Verification items for the finished model (mm, model axes). A direction names the side the tool comes from. Give positions to 0.01 mm unless a question says otherwise; leave off trailing zeros. Order: outer loops, then holes, each group sorted by start corner. A loop starts at its lowest first (then second) coordinate and runs counter-clockwise, first axis right, second up.
from build123d import *

# Parameters (mm, degrees)
CHAMFER2_SIZE      = 1
CUT_EXTRUDE1_START = -10
SKETCH2_R          = 31.378818645
CUT_EXTRUDE1_DEPTH = 10
CHAMFER3_SIZE      = 1
CUT_EXTRUDE2_REACH = 52.21
SKETCH4_R          = 2
SCALE_1_SCALE      = 1.875


with BuildPart() as part:
    # Sketch1 → Revolve2 (revolve)
    with BuildSketch(Plane.XY, mode=Mode.PRIVATE) as revolve2_sk:
        with BuildLine():
            Line((6, 0), (6, 37))
            Line((6, 37), (24, 37))
            Line((24, 37), (24, 32))
            Line((24, 32), (14, 32))
            ThreePointArc((14, 32), (12.392227943, 28.198889706), (15, 25))
            Line((15, 25), (20, 25))
            Line((20, 25), (20, 15))
            Line((20, 15), (10, 15))
            Line((10, 15), (10, 12))
            Line((10, 12), (14, 12))
            Line((14, 12), (14, 0))
            Line((14, 0), (6, 0))
        make_face()
    revolve(revolve2_sk.sketch.rotate(Axis((0, 0, 0), (0, 1, 0)), 90), axis=Axis((0, 0, 0), (0, 1, 0)))

    # Chamfer2
    chamfer2_edges = [part.edges().sort_by_distance(p)[0] for p in [
        (0, 0, 14),
    ]]
    chamfer(chamfer2_edges, length=CHAMFER2_SIZE)

    # Sketch2 → Cut-Extrude1 (cut)
    with BuildSketch(Plane(origin=(0, 25, 0), x_dir=(1, 0, 0), z_dir=(0, 1, 0)).offset(CUT_EXTRUDE1_START)):
        Circle(SKETCH2_R)
        Polygon((20, 0), (10, 17.320508076), (-10, 17.320508076), (-20, 0), (-10, -17.320508076), (10, -17.320508076), align=None, mode=Mode.SUBTRACT)
    extrude(amount=CUT_EXTRUDE1_DEPTH, mode=Mode.SUBTRACT)

    # Sketch3 → Cut-Revolve1 (revolve, cut)
    with BuildSketch(Plane.XY, mode=Mode.PRIVATE) as cut_revolve1_sk:
        with BuildLine():
            Line((-20, 24), (-20, 25))
            Line((-20, 25), (-16.614510602, 25))
            ThreePointArc((-16.614510602, 25), (-18.356765058, 24.667614757), (-20, 24))
        make_face()
    revolve(cut_revolve1_sk.sketch.rotate(Axis((0, 0, 0), (0, 1, 0)), 270), axis=Axis((0, 0, 0), (0, 1, 0)), mode=Mode.SUBTRACT)

    # Chamfer3
    chamfer3_edges = [part.edges().sort_by_distance(p)[0] for p in [
        (0, 37, 24),
    ]]
    chamfer(chamfer3_edges, length=CHAMFER3_SIZE)

    # Sketch4 → Cut-Extrude2 (cut, up to next)
    with BuildSketch(Plane(origin=(0, 37, 0), x_dir=(1, 0, 0), z_dir=(0, 1, 0)), mode=Mode.PRIVATE) as cut_extrude2_sk1:
        with Locations(Location((17, 0, 0), (0, 0, 270))):
            Circle(SKETCH4_R)
    cut_extrude2_tool1 = extrude(cut_extrude2_sk1.sketch, amount=-CUT_EXTRUDE2_REACH, mode=Mode.PRIVATE) & part.part
    # Sketch4 → Cut-Extrude2 (cut, up to next)
    with BuildSketch(Plane(origin=(0, 37, 0), x_dir=(1, 0, 0), z_dir=(0, 1, 0)), mode=Mode.PRIVATE) as cut_extrude2_sk2:
        with Locations(Location((-17, 0, 0), (0, 0, 90))):
            Circle(SKETCH4_R)
    cut_extrude2_tool2 = extrude(cut_extrude2_sk2.sketch, amount=-CUT_EXTRUDE2_REACH, mode=Mode.PRIVATE) & part.part
    add(cut_extrude2_tool1.solids().sort_by_distance((17, 37, 0))[0], mode=Mode.SUBTRACT)
    add(cut_extrude2_tool2.solids().sort_by_distance((-17, 37, 0))[0], mode=Mode.SUBTRACT)


with BuildPart() as part_1:
    # Scale 1: scaled about (-3.12e-07, 22.102096906, 1.9e-08)
    add(part.part.scale(SCALE_1_SCALE).moved(Location((2.73e-07, -19.339334793, -1.7e-08))))


solid = part_1.part
(1) Release check for a two-part mould opening along X. For faces 1 (the flat face through (-27.99, 17.94, -16.47)), 2 (the flat face through (19, 40.661, -19)), 3 (the cylindrical face through (35.593, 45.414, -0.488)), 4 (the cylindrical face through (43.93, 44.36, 9.76)) record: pulls with the +X half, pulls with the -X half, needs draft (parallel to the pull), parting line crosses it, or undercut.
Solved:
face 1: pulls with the -X half
face 2: needs draft
face 3: undercut
face 4: parting line crosses it
(2) Section check A-A, the plane y = -0.5. Enter the section's corners in (x, z).
Solved:
outline: circle Ø52.5 at (0, 0); hole circle Ø22.5 at (0, 0)
(3) Go/stop test with flat-tipped pins: pin 1 (8 mm diameter, centred on x = 17.5, y = 4, fed in from +Z); pin 2 (8 mm diameter, centred on y = 21.5, z = 32, fed in from -X); pin 3 (5 mm diameter, centred on y = 38, z = -34.5, fed in from -X); pin 4 (19.5 mm diameter, centred on x = 2, z = -5, fed in from -Y). Record where each tip stops, or that it passes through.
Solved:
pin 1: stops at z = 22.46
pin 2: stops at x = -21.33
pin 3: passes through
pin 4: stops at y = -19.34
(4) Scan lines: line 1 (X direction, y = 44.5, z = 0) (3 decimals); line 2 (Z direction, x = -0.5, y = -6); line 3 (X direction, y = -4, z = 0). Record each from-to range of solid material in increasing order.
Solved:
line 1: x = -45 to -35.625, -28.125 to -11.25, 11.25 to 28.125, 35.625 to 45
line 2: z = -26.25 to -11.24, 11.24 to 26.25
line 3: x = -26.25 to -11.25, 11.25 to 26.25
(5) Set-up check for faces 5 (the cylindrical face through (11.41, 5.93, 14.88)), 6 (the cylindrical face through (-28.214, 45.414, 0.813)), 7 (the flat face through (0, 18, 32.476)), 8 (the cylindrical face through (15.973, -7.296, 20.831)), 9 (the flat face through (28.256, 17.945, -16.011)): record each of +Z, -Z, +X, -X, +Y, -Y from which the full face is reachable in a straight line by a thin tool's end or side.
Solved:
face 5: none
face 6: +Y
face 7: +Z, +X, -X, -Y
face 8: -Y
face 9: -Z, +X, -Y
